```python
from build123d import *

# Parameters (mm, degrees)
SKETCH_1_W          = 2
SKETCH_1_H          = 180
EXTRUDE_1_DEPTH     = 50
SKETCH_2_R          = 2
CUT_EXTRUDE_1_DEPTH = 20
SKETCH_3_R          = 2
CUT_EXTRUDE_2_DEPTH = 10
SKETCH_4_W          = 190.004489292
SKETCH_4_H          = 85.174426234
CUT_EXTRUDE_3_DEPTH = 10


with BuildPart() as part:
    # 草图1 → 凸台-拉伸1 (new body)
    with BuildSketch(Plane.XY):
        Rectangle(SKETCH_1_W, SKETCH_1_H)
    extrude(amount=EXTRUDE_1_DEPTH)

    # 草图2 → 切除-拉伸1 (cut)
    with BuildSketch(Plane(origin=(1, 0, 0), x_dir=(0, 0, -1), z_dir=(1, 0, 0))):
        with Locations((-25, -40)):
            Circle(SKETCH_2_R)
    extrude(amount=-CUT_EXTRUDE_1_DEPTH, mode=Mode.SUBTRACT)

    # 草图3 → 切除-拉伸2 (cut)
    with BuildSketch(Plane(origin=(1, 0, 0), x_dir=(0, 0, -1), z_dir=(1, 0, 0))):
        with Locations((-25, 50)):
            Circle(SKETCH_3_R)
    extrude(amount=-CUT_EXTRUDE_2_DEPTH, mode=Mode.SUBTRACT)

    # 草图4 → 切除-拉伸3 (cut)
    with BuildSketch(Plane.ZY.offset(1)):
        with Locations((56.530917404, -102.587213117)):
            Rectangle(SKETCH_4_W, SKETCH_4_H)
    extrude(amount=-CUT_EXTRUDE_3_DEPTH, mode=Mode.SUBTRACT)


solid = part.part
```
Build history of the part. All positions in model axes, mm. Give positions to 0.01 mm unless a question says otherwise; leave off trailing zeros. Loops run counter-clockwise (first coordinate to the right, second up) from the corner with the lowest first, then second, coordinate; pieces in that order, holes last. Notation, with made-up numbers: (-1.75, 60.25) - (6.25, 60.25) arc R20 ccw to (6.25, 69.25) - close; hole circle Ø5 at (3, 46.25). An arc over 180 degrees is marked (long way). Use a Markdown table: item, result.
(1) Drop a flat-ended pin along its axis: pin 1 Ø6.5 at (y, z) = (50, 25) entering from +X. Give the stop position or say it passes through.
Taken from the geometry:
| item | result |
|---|---|
| pin 1 | x = 1 |
(2) Band-saw the part on A-A (y = 50). Give the cut face in (x, z).
Taken from the geometry:
| item | result |
|---|---|
| outline | (-1, 0) - (1, 0) - (1, 23) - (-1, 23) - close; (-1, 27) - (1, 27) - (1, 50) - (-1, 50) - close |
(3) Wall check: line 1 along Y through (x, z) = (-0.2, 25). Give the ranges that are in metal, low to high.
Taken from the geometry:
| item | result |
|---|---|
| line 1 | -60 to -42, -38 to 48, 52 to 90 |
(4) Pull direction Y, two halves, no side cores. Call faces 1 (the face through (0, -42, 25)), 2 (the face through (-1, 14, 25)): +Y half, -Y half, draft (parallel to the pull), parting line (faces both ways), or undercut.
Taken from the geometry:
| item | result |
|---|---|
| face 1 | undercut |
| face 2 | draft |
(5) Band-saw the part on B-B (z = 25). Give the cut face in (x, y).
Taken from the geometry:
| item | result |
|---|---|
| outline | (-1, -60) - (1, -60) - (1, -42) - (-1, -42) - close; (-1, -38) - (1, -38) - (1, 48) - (-1, 48) - close; (-1, 52) - (1, 52) - (1, 90) - (-1, 90) - close |
